The listing builds one solid part. Answer for the finished solid, in the listing's coordinates (mm). A direction names the side the tool comes from. Give positions to 0.01 mm unless a question says otherwise; leave off trailing zeros. Loops run counter-clockwise (first coordinate to the right, second up) from the corner with the lowest first, then second, coordinate; pieces in that order, holes last. Notation, with made-up numbers: (9.5, -6.5) - (56.5, -6.5) arc R22 ccw to (56.5, 12.5) - close; hole circle Ø9 at (-35, 65.5). An arc over 180 degrees is marked (long way). Write each question's results on one line, items separated by ' | '.
from build123d import *

# Parameters (mm, degrees)
HOLE_WIZARD_M2_1_D           = 2.4
HOLE_WIZARD_M2_1_CBORE_D     = 5
HOLE_WIZARD_M2_1_CBORE_DEPTH = 7


with BuildPart() as part:
    # 草图1 → 旋转1 (revolve)
    with BuildSketch(Plane.XY, mode=Mode.PRIVATE) as revolve_1_sk:
        with BuildLine():
            Line((0, -11), (0, -15.5))
            ThreePointArc((0, -15.5), (8.144809073, -14.009581241), (15.234037604, -9.731485667))
            ThreePointArc((15.234037604, -9.731485667), (15.718094855, -9.086559789), (15.908120336, -8.302894602))
            Line((15.908120336, -8.302894602), (16, -5.671805268))
            Line((16, -5.671805268), (9.974317744, -5.671805268))
            ThreePointArc((9.974317744, -5.671805268), (9.503140374, -5.789766785), (9.143124599, -6.115821496))
            ThreePointArc((9.143124599, -6.115821496), (5.182951068, -9.702423317), (0, -11))
        make_face()
    revolve(revolve_1_sk.sketch.rotate(Axis((0, -11, 0), (0, -1, 0)), 90), axis=Axis((0, -11, 0), (0, -1, 0)))

    # M2 六角头螺栓的柱形沉头孔1 (through all)
    with Locations(Plane.XZ.offset(15.671805268)):
        with Locations((-14.25, 0), (0, -14.25), (14.25, 0), (0, 14.25)):
            CounterBoreHole(HOLE_WIZARD_M2_1_D / 2, HOLE_WIZARD_M2_1_CBORE_D / 2, HOLE_WIZARD_M2_1_CBORE_DEPTH)


solid = part.part
Item 1: For a pull along Z with two mould halves and no side action, classify faces 1 (the face through (15.555, -7.554, -3.454)), 2 (the face through (-12.9, -8.672, 0)), 3 (the face through (10.4, -5.672, -0.2)), 4 (the face through (13.105, -7.151, 0.36)) as released by +Z, released by -Z, zero draft, split by the parting line, or undercut.
Values found:
face 1: split by the parting line | face 2: undercut | face 3: zero draft | face 4: undercut
Item 2: Flat-ended cylindrical pins translate along their axes: P1, Ø2, axis at x = 1, y = -14, coming from the -Z side; P2, Ø3, axis at y = -7, z = -5, coming from the -X side; P3, Ø6, axis at x = 5, z = -7, coming from the -Y side; P4, Ø3, axis at x = 0, z = -14.25, coming from the +Y side. Find the tip coordinate at first contact, or state that the pin passes through.
Values found:
P1: stops at z = -10.38 | P2: stops at x = -15.57 | P3: stops at y = -14.81 | P4: stops at y = -5.67
Item 3: Find the intervals of material crossed by line 1 along Z through (x, y) = (0, -11.2); line 2 along Z through (x, y) = (13.5, -7); line 3 along X through (y, z) = (-7, -5.5), in increasing order. Write a range as [from, to].
Values found:
line 1: z = [-11.75, 11.75] | line 2: z = [-8.5, -0.94], [0.94, 8.5] | line 3: x = [-14.98, -6.46], [6.46, 14.98]
Item 4: For faces 5 (the face through (11.75, -10.1, 0.08)), 6 (the face through (-15.395, -7.151, 0.36)), determine the directions among +Z, -Z, +X, -X, +Y, -Y from which every point of the face is accessible in a straight line to the end or side of a thin tool.
Values found:
face 5: -Y | face 6: +Y, -Y
Item 5: A cutting plane is placed at A-A, the plane x = 0. Determine the outline of the cut face in (y, z).
Values found:
outline: (-12.27, -11.75) - (-8.67, -11.75) - (-8.67, -13.05) - (-5.67, -13.05) - (-5.67, -9.97) arc R1 ccw to (-6.12, -9.14) arc R11 cw to (-6.12, 9.14) arc R1 ccw to (-5.67, 9.97) - (-5.67, 13.05) - (-8.67, 13.05) - (-8.67, 11.75) - (-12.27, 11.75) arc R23 ccw to start; (-8.67, -15.86) arc R2 ccw to (-8.3, -15.91) - (-5.67, -16) - (-5.67, -15.45) - (-8.67, -15.45) - close; (-8.67, 15.45) - (-5.67, 15.45) - (-5.67, 16) - (-8.3, 15.91) arc R2 ccw to (-8.67, 15.86) - close
Item 6: A cutting plane is placed at B-B, the plane y = -13. Determine the outline of the cut face in (x, z).
Values found:
outline: circle Ø20.86 at (0, 0)
